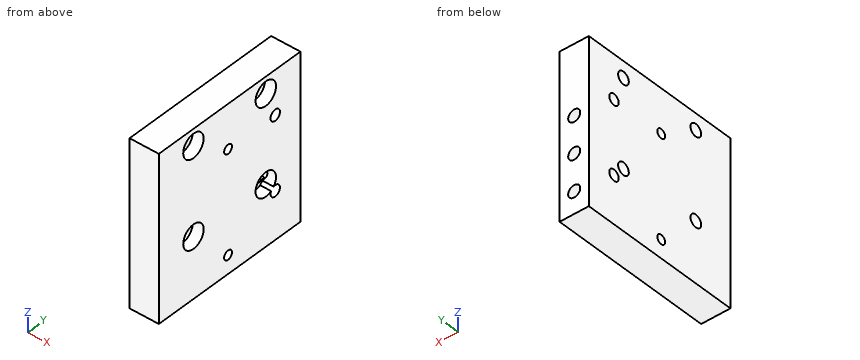
from build123d import *

# Parameters (mm, degrees)
SKETCH_1_W                                        = 45
SKETCH_1_H                                        = 45
BOSS_EXTRUDE_1_DEPTH                              = 8
M3_HEX_SOCKET_CAP_SCREW_COUNTERBORE_1_D           = 3.4
M3_HEX_SOCKET_CAP_SCREW_COUNTERBORE_1_CBORE_D     = 6.5
M3_HEX_SOCKET_CAP_SCREW_COUNTERBORE_1_CBORE_DEPTH = 3
LINEAR_PATTERN_1_COUNT                            = 2
LINEAR_PATTERN_1_PITCH                            = 23
LINEAR_PATTERN_2_COUNT                            = 2
LINEAR_PATTERN_2_PITCH                            = 24
LINEAR_PATTERN_2_COPY_1_D                         = 3.4
LINEAR_PATTERN_2_COPY_1_CBORE_D                   = 6.5
LINEAR_PATTERN_2_COPY_1_CBORE_DEPTH               = 3
LINEAR_PATTERN_5_COUNT                            = 3
LINEAR_PATTERN_5_PITCH                            = 10
M3_TAPPED_HOLE_1_D                                = 2.5
LINEAR_PATTERN_6_COUNT                            = 2
LINEAR_PATTERN_6_PITCH                            = 28
F_3_0_3_HOLE_1_D                                  = 3
LINEAR_PATTERN_8_COUNT                            = 2
LINEAR_PATTERN_8_PITCH                            = 20


with BuildPart() as part:
    # Sketch 1 → Boss-Extrude 1 (new body)
    with BuildSketch(Plane(origin=(0, 0, 0), x_dir=(0, 0, -1), z_dir=(1, 0, 0))):
        Rectangle(SKETCH_1_W, SKETCH_1_H)
    extrude(amount=BOSS_EXTRUDE_1_DEPTH)

    # M3 Hex Socket Cap Screw Counterbore 1 (through all)
    with Locations(Plane(origin=(8, 0, 0), x_dir=(0, 0, -1), z_dir=(1, 0, 0))):
        with Locations((-18, 11.5)):
            m3_hex_socket_cap_screw_counterbore_1 = CounterBoreHole(M3_HEX_SOCKET_CAP_SCREW_COUNTERBORE_1_D / 2, M3_HEX_SOCKET_CAP_SCREW_COUNTERBORE_1_CBORE_D / 2, M3_HEX_SOCKET_CAP_SCREW_COUNTERBORE_1_CBORE_DEPTH)

    # Linear Pattern 1: M3 Hex Socket Cap Screw Counterbore 1 ×2
    with Locations(*[(0, -i * LINEAR_PATTERN_1_PITCH, 0) for i in range(1, LINEAR_PATTERN_1_COUNT)]):
        add(m3_hex_socket_cap_screw_counterbore_1, mode=Mode.SUBTRACT)

    # Linear Pattern 2: M3 Hex Socket Cap Screw Counterbore 1 ×2
    with Locations(*[(0, 0, -i * LINEAR_PATTERN_2_PITCH) for i in range(1, LINEAR_PATTERN_2_COUNT)]):
        add(m3_hex_socket_cap_screw_counterbore_1, mode=Mode.SUBTRACT)

    # Linear Pattern 2 copy 1 (through all)
    with Locations(Plane(origin=(8, -23, -24), x_dir=(0, 0, -1), z_dir=(1, 0, 0))):
        with Locations((-18, 11.5)):
            CounterBoreHole(LINEAR_PATTERN_2_COPY_1_D / 2, LINEAR_PATTERN_2_COPY_1_CBORE_D / 2, LINEAR_PATTERN_2_COPY_1_CBORE_DEPTH)

    # Sketch 6 → M4 Tapped Hole 1 (revolve, cut)
    with BuildSketch(Plane(origin=(4, 22.5, -16.5), x_dir=(0, 0, 1), z_dir=(1, 0, 0))):
        Polygon((0, 0), (0, 11.091420021), (1.65, 10.1), (1.65, 0), align=None)
    m4_tapped_hole_1 = revolve(axis=Axis((4, 28.85, -16.5), (0, -1, 0)), mode=Mode.SUBTRACT)

    # Linear Pattern 5: M4 Tapped Hole 1 ×3
    with Locations(*[(0, 0, i * LINEAR_PATTERN_5_PITCH) for i in range(1, LINEAR_PATTERN_5_COUNT)]):
        add(m4_tapped_hole_1, mode=Mode.SUBTRACT)

    # M3 Tapped Hole 1 (through all)
    with Locations(Plane(origin=(8, 0, 0), x_dir=(0, 0, -1), z_dir=(1, 0, 0))):
        with Locations((17.5, -0.5)):
            m3_tapped_hole_1 = Hole(M3_TAPPED_HOLE_1_D / 2)

    # Linear Pattern 6: M3 Tapped Hole 1 ×2
    with Locations(*[(0, 0, i * LINEAR_PATTERN_6_PITCH) for i in range(1, LINEAR_PATTERN_6_COUNT)]):
        add(m3_tapped_hole_1, mode=Mode.SUBTRACT)

    # Ø3.0 (3) Hole 1 (through all)
    with Locations(Plane(origin=(8, 0, 0), x_dir=(0, 0, -1), z_dir=(1, 0, 0))):
        with Locations((-10.5, 14.5)):
            f_3_0_3_hole_1 = Hole(F_3_0_3_HOLE_1_D / 2)

    # Linear Pattern 8: Ø3.0 (3) Hole 1 ×2
    with Locations(*[(0, 0, -i * LINEAR_PATTERN_8_PITCH) for i in range(1, LINEAR_PATTERN_8_COUNT)]):
        add(f_3_0_3_hole_1, mode=Mode.SUBTRACT)


solid = part.part
Verification items for the finished model (mm, model axes). Coordinates: 2 decimals unless noted, no trailing zeros. Loops run counter-clockwise (first coordinate to the right, second up) from the corner with the lowest first, then second, coordinate; pieces in that order, holes last. Notation, with made-up numbers: (-7, 7.25) -> (25, 7.25) arc R30 cw to (25, 35.25) -> close; hole circle Ø7 at (64, 73.5). An arc over 180 degrees is marked (long way). Answer as a JSON object with one key per item and string values. Group by question number.
Item 1: Scan lines: probe 1 along Y at (x, z) = (7.1, 18); probe 2 along Y at (x, z) = (6.25, 10.5); probe 3 along Y at (x, z) = (6.75, -17.5). Record each from-to range of solid material in increasing order.
Item 2: Sectioned sample at A-A on x = 1.75. State how many separate pieces and enclosed holes the cut face has, plus the area to 3 significant figures.
Item 3: Sectioned sample at C-C on z = -6.5. Record the boundary of the cut face in (x, y), plus the area to 3 significant figures.
Item 4: Depth check by flat-ended pin: pin 1 (7.5 mm diameter, centred on y = -11.5, z = 18, fed in from -X); pin 2 (5.5 mm diameter, centred on y = 11.5, z = 18, fed in from +X); pin 3 (3 mm diameter, centred on y = -11.5, z = -6, fed in from +X). Enter the tip coordinate at first touch or a pass-through.
Item 5: Sectioned sample at B-B on z = 18. Record the boundary of the cut face in (x, y), plus the area to 3 significant figures.
Evaluation:
{
 "1": {"probe 1": "y = -22.5 to -14.75, -8.25 to 8.25, 14.75 to 22.5", "probe 2": "y = -22.5 to -1.75, 0.75 to 13, 16 to 22.5", "probe 3": "y = -22.5 to -1.75, 0.75 to 22.5"},
 "2": {"separate pieces": "1", "enclosed holes": "8", "area": "1,960 mm²"},
 "3": {"outline": "(0, -22.5) -> (8, -22.5) -> (8, -14.71) -> (5, -14.71) -> (5, -13.12) -> (0, -13.12) -> close; (0, -9.88) -> (5, -9.88) -> (5, -8.29) -> (8, -8.29) -> (8, 8.29) -> (5, 8.29) -> (5, 9.88) -> (0, 9.88) -> close; (0, 13.12) -> (2.35, 13.12) -> (2.35, 22.5) -> (0, 22.5) -> close; (5.65, 14.71) -> (8, 14.71) -> (8, 22.5) -> (5.65, 22.5) -> close", "area": "259 mm²"},
 "4": {"pin 1": "stops at x = 0", "pin 2": "stops at x = 5", "pin 3": "passes through"},
 "5": {"outline": "(0, -22.5) -> (8, -22.5) -> (8, -14.75) -> (5, -14.75) -> (5, -13.2) -> (0, -13.2) -> close; (0, -9.8) -> (5, -9.8) -> (5, -8.25) -> (8, -8.25) -> (8, 8.25) -> (5, 8.25) -> (5, 9.8) -> (0, 9.8) -> close; (0, 13.2) -> (5, 13.2) -> (5, 14.75) -> (8, 14.75) -> (8, 22.5) -> (0, 22.5) -> close", "area": "287 mm²"}
}
